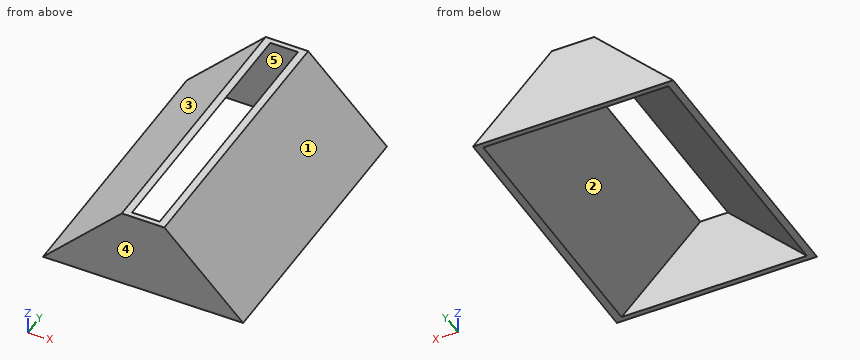
from build123d import *

# Parameters (mm, degrees)
BOSS_EXTRUDE1_DEPTH = 520
SHELL1_T            = -10


with BuildPart() as part:
    # Sketch1 → Boss-Extrude1 (new body)
    with BuildSketch(Plane(origin=(0, 0, 0), x_dir=(1, 0, 0), z_dir=(0, 1, 0))):
        Polygon((0, 0), (40, 0), (188, 150), (0, 150), align=None)
    boss_extrude1 = extrude(amount=BOSS_EXTRUDE1_DEPTH)

    # Mirror1: Boss-Extrude1 across plane
    add(boss_extrude1.mirror(Plane(origin=(0, 520, 0), x_dir=(0, 0, 1), z_dir=(1, 0, 0))))

    # Shell1
    shell1_openings = [part.faces().sort_by_distance(p)[0] for p in [
        (0, 260, -150),
        (0, 260, 0),
    ]]
    offset(amount=SHELL1_T, openings=shell1_openings, kind=Kind.INTERSECTION)


solid = part.part
Can you work these out from the model? Positions are in its coordinate system, mm. Face numbers are marked on the shaded views. A direction names the side the tool comes from. Round coordinates to 2 decimals unless told otherwise and drop trailing zeros. Order: outer loops, then holes, each group sorted by start corner. A loop starts at its lowest first (then second) coordinate and runs counter-clockwise, first axis right, second up. Notation, with made-up numbers: (30, 11.5) -> (76, 11.5) arc R27 ccw to (76, 50.5) -> close; hole circle Ø8 at (62.25, 4.5). An arc over 180 degrees is marked (long way). Write each question's results on one line, items separated by ' | '. Start each with the question number.
Item 1: If we section it at A-A, the plane y = 266.5: Write out the boundary of the cut face in (x, z), then the cut area to 3 significant figures.
Item 2: If we section it at D-D, the plane x = 58.5: Write out the boundary of the cut face in (y, z), then the cut area to 3 significant figures.
Item 3: If we section it at C-C, the plane z = -43: Write out the boundary of the cut face in (x, y).
Item 4: Please list where these lines run through material, in increasing order: L1, parallel to Y at x = -126.5, z = -134; L2, parallel to X at y = 469, z = -109; L3, parallel to X at y = 39, z = -88.
Item 5: Thinking about a two-plate mould opening in Y: for the marked faces 3, 4 and 5, which applies, +Y half, -Y half, draft (parallel to the pull), parting line (faces both ways), or undercut?
Item 6: If we section it at B-B, the plane x = 13.5: Write out the boundary of the cut face in (y, z).
Item 7: Will these pins go through, and if not, where does the flat tip stop? pin 1 (10 mm diameter, centred on y = 398.5, z = -23.5, fed in from -X); pin 2 (3 mm diameter, centred on x = 73.5, y = 442, fed in from +Z); pin 3 (4 mm diameter, centred on y = 432, z = -127.5, fed in from -X).
Item 8: Which directions (+Z, -Z, +X, -X, +Y, -Y) give clear straight access to the entire face, cutting with the end or side of a thin tool? Please do the marked faces 1 and 2.
Results:
1) outline: (-188, -150) -> (-173.95, -150) -> (-25.95, 0) -> (-40, 0) -> close; (25.95, 0) -> (173.95, -150) -> (188, -150) -> (40, 0) -> close | area: 4,210 mm2
2) outline: (0, -150) -> (10, -150) -> (10, -32.99) -> (510, -32.99) -> (510, -150) -> (520, -150) -> (520, -18.75) -> (0, -18.75) -> close | area: 9,740 mm2
3) outline: (-82.43, 0) -> (82.43, 0) -> (82.43, 520) -> (-82.43, 520) -> close; hole (-68.38, 10) -> (68.38, 10) -> (68.38, 510) -> (-68.38, 510) -> close
4) L1: y = 0 to 10, 510 to 520 | L2: x = -147.55 to -133.5, 133.5 to 147.55 | L3: x = -126.83 to -112.78, 112.78 to 126.83
5) face 3: draft | face 4: -Y half | face 5: undercut
6) outline: (0, -150) -> (10, -150) -> (10, 0) -> (0, 0) -> close; (510, -150) -> (520, -150) -> (520, 0) -> (510, 0) -> close
7) pin 1: stops at x = -68.12 | pin 2: stops at z = -32.43 | pin 3: stops at x = -167.77
8) face 1: +Z, +X, +Y, -Y | face 2: -Z
